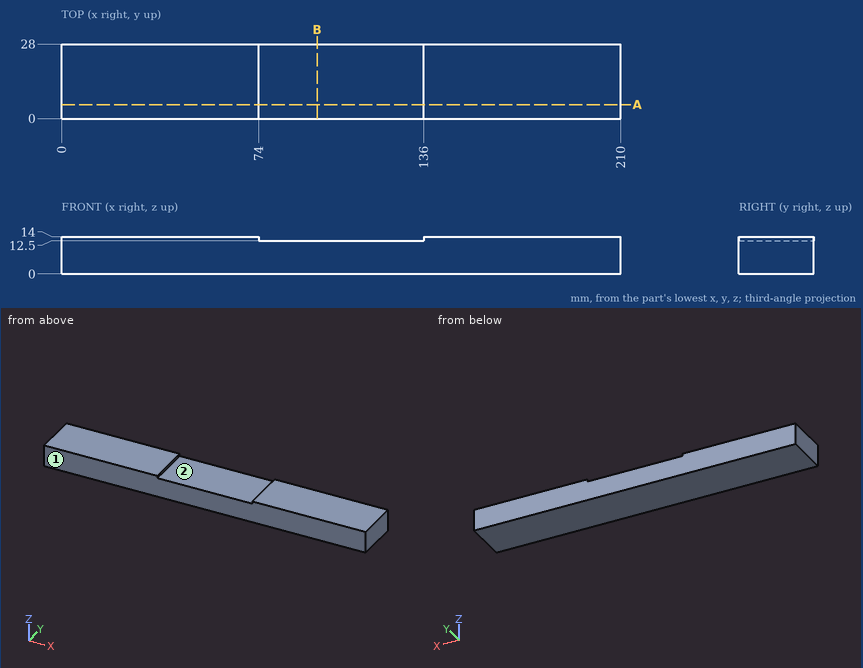
Here's the drawing with two shaded views (mm, measured from the low corner). I have some questions. Give positions to 0.01 mm unless a question says otherwise; leave off trailing zeros. Loops run counter-clockwise (first coordinate to the right, second up) from the corner with the lowest first, then second, coordinate; pieces in that order, holes last. Notation, with made-up numbers: (-18, 78) -> (-14, 78) arc R37 ccw to (-14, 116) -> close; hole circle Ø7 at (11.25, -28). An arc over 180 degrees is marked (long way). One line per item, written item: value.
Q1. Suppose I cut it at A-A on y = 5.25. Please give me the cut outline in (x, z).
Answers follow:
outline: (0, 0) -> (210, 0) -> (210, 14) -> (136, 14) -> (136, 12.5) -> (74, 12.5) -> (74, 14) -> (0, 14) -> close
Q2. We'd pull the mould along X, two halves only. Please class the marked faces 1 and 2: pulls with the +X half, pulls with the -X half, needs draft (parallel to the pull), parting line crosses it, or undercut.
Answers follow:
face 1: needs draft
face 2: undercut
Q3. If I drill on line 1 along X through (y, z) = (5, 13); line 2 along Z through (x, y) = (121, 16), over which ranges is the centre line in solid material (lowest first)?
Answers follow:
line 1: 0 to 74, 136 to 210
line 2: 0 to 12.5
Q4. I'm going to push a flat-ended pin straight in: pin 1 Ø1.2 at (y, z) = (17.5, 13.5) entering from -X. Where does the tip first touch, or does it pass through?
Answers follow:
pin 1: x = 0
Q5. Suppose I cut it at B-B on x = 96. Please give me the cut outline in (y, z), then the cut area to 3 significant figures.
Answers follow:
outline: (0, 0) -> (28, 0) -> (28, 12.5) -> (0, 12.5) -> close
area: 350 mm^2
